Geometry: final body of the model. Coordinates: model frame, mm. Face numbers are marked on the shaded views. Give positions to 0.01 mm unless a question says otherwise; leave off trailing zeros. Loops run counter-clockwise (first coordinate to the right, second up) from the corner with the lowest first, then second, coordinate; pieces in that order, holes last.
from build123d import *

# Parameters (mm, degrees)
BALL_FACE_1_SKETCH_R       = 25
BALL_FACE_CUT_1_DEPTH      = 7.5
BALL_FACE_2_SKETCH_R       = 25
BALL_FACE_CUT_2_DEPTH      = 7.5
KEYED_BORE_20_REACH        = 210.153
SMALL_END_FLAT_CUT_1_REACH = 216.934
SMALL_START                = -9
SMALL_END_FLAT_CUT_2_REACH = 216.934
SMALL_START_2              = 9
SMALL_END_EYE_CUT_REACH    = 208.893
SMALL_END_EYE_SKETCH_R     = 9
HOLE_8_CUT_REACH           = 207.934
HOLE_8_CUT_END_RADIUS      = 25
HOLE_8_SKETCH_R            = 4


with BuildPart() as part:
    # Lever Profile Sketch → Lever Body Revolve (revolve)
    with BuildSketch(Plane(origin=(0, 0, 0), x_dir=(1, 0, 0), z_dir=(0, 1, 0)), mode=Mode.PRIVATE) as lever_body_revolve_sk:
        with BuildLine():
            Line((168.522248412, -10), (33.541019662, -10))
            ThreePointArc((33.541019662, -10), (25.376053853, -11.742581416), (18.633899812, -16.666666667))
            ThreePointArc((18.633899812, -16.666666667), (-8.920552244, -23.354308974), (-25, 0))
            Line((-25, 0), (203.66060556, 0))
            ThreePointArc((203.66060556, 0), (193.547273819, -15.542644572), (175.240158467, -12.592592593))
            ThreePointArc((175.240158467, -12.592592593), (172.122659912, -10.670635765), (168.522248412, -10))
        make_face()
    revolve(lever_body_revolve_sk.sketch.rotate(Axis((248.139692176, 0, 0), (-1, 0, 0)), 180), axis=Axis((248.139692176, 0, 0), (-1, 0, 0)))

    # Ball Face 1 Sketch → Ball Face Cut 1 (cut)
    with BuildSketch(Plane.XY.offset(25)):
        Circle(BALL_FACE_1_SKETCH_R)
    extrude(amount=-BALL_FACE_CUT_1_DEPTH, mode=Mode.SUBTRACT)


with BuildPart() as ball_face_cut_1_kept_piece:
    # of the separate pieces the step leaves, the one the design keeps (ball_face_cut_1_pieces_kept)
    add(part.part.solids().sort_by_distance((175.240158467, 0, -12.592592593))[0])

    # Ball Face 2 Sketch → Ball Face Cut 2 (cut)
    with BuildSketch(Plane.XY.offset(-25)):
        Circle(BALL_FACE_2_SKETCH_R)
    extrude(amount=BALL_FACE_CUT_2_DEPTH, mode=Mode.SUBTRACT)

    # Keyed Bore Sketch → Keyed Bore _20 (cut, up to next)
    with BuildSketch(Plane(origin=(0, 0, -17.5), x_dir=(-1, 0, 0), z_dir=(0, 0, -1)), mode=Mode.PRIVATE) as keyed_bore_20_sk1:
        with BuildLine():
            Line((-13, 2), (-9.797958971, 2))
            ThreePointArc((-9.797958971, 2), (10, 0), (-9.797958971, -2))
            Line((-9.797958971, -2), (-13, -2))
            Line((-13, -2), (-13, 2))
        make_face()
    keyed_bore_20_tool1 = extrude(keyed_bore_20_sk1.sketch, amount=-KEYED_BORE_20_REACH, mode=Mode.PRIVATE) & ball_face_cut_1_kept_piece.part
    add(keyed_bore_20_tool1.solids().sort_by_distance((0.430928, 0, -17.5))[0], mode=Mode.SUBTRACT)

    # Small End Flats Sketch → Small End Flat Cut 1 (cut, up to next)
    with BuildSketch(Plane.XY.offset(SMALL_START), mode=Mode.PRIVATE) as small_end_flat_cut_1_sk1:
        with BuildLine():
            Line((170.41252875, 5), (148.66060556, 5))
            Line((148.66060556, 5), (148.66060556, -5))
            Line((148.66060556, -5), (170.41252875, -5))
            ThreePointArc((170.41252875, -5), (203.66060556, 0), (170.41252875, 5))
        make_face()
    small_end_flat_cut_1_tool1 = extrude(small_end_flat_cut_1_sk1.sketch, amount=-SMALL_END_FLAT_CUT_1_REACH, mode=Mode.PRIVATE) & ball_face_cut_1_kept_piece.part
    add(small_end_flat_cut_1_tool1.solids().sort_by_distance((181.469026, 0, -9))[0], mode=Mode.SUBTRACT)

    # Sketch11_2 → Small End Flat Cut 2 (cut, up to next)
    with BuildSketch(Plane.XY.offset(SMALL_START_2), mode=Mode.PRIVATE) as small_end_flat_cut_2_sk1:
        with BuildLine():
            Line((170.41252875, 5), (148.66060556, 5))
            Line((148.66060556, 5), (148.66060556, -5))
            Line((148.66060556, -5), (170.41252875, -5))
            ThreePointArc((170.41252875, -5), (203.66060556, 0), (170.41252875, 5))
        make_face()
    small_end_flat_cut_2_tool1 = extrude(small_end_flat_cut_2_sk1.sketch, amount=SMALL_END_FLAT_CUT_2_REACH, mode=Mode.PRIVATE) & ball_face_cut_1_kept_piece.part
    add(small_end_flat_cut_2_tool1.solids().sort_by_distance((181.469026, 0, 9))[0], mode=Mode.SUBTRACT)

    # Small End Eye Sketch → Small End Eye Cut (cut, up to next)
    with BuildSketch(Plane.XY.offset(9), mode=Mode.PRIVATE) as small_end_eye_cut_sk1:
        with Locations((186.66060556, 0)):
            Circle(SMALL_END_EYE_SKETCH_R)
    small_end_eye_cut_tool1 = extrude(small_end_eye_cut_sk1.sketch, amount=-SMALL_END_EYE_CUT_REACH, mode=Mode.PRIVATE) & ball_face_cut_1_kept_piece.part
    add(small_end_eye_cut_tool1.solids().sort_by_distance((186.660606, 0, 9))[0], mode=Mode.SUBTRACT)

    # Hole _8 Cut: up to this sphere (the profile starts inside it)
    hole_8_cut_end = Location((0, 0, 0)) * Sphere(HOLE_8_CUT_END_RADIUS, mode=Mode.PRIVATE)
    # Hole _8 Sketch → Hole _8 Cut (cut, up to the surface)
    with BuildSketch(Plane(origin=(0, 0, 0), x_dir=(0, 0, -1), z_dir=(1, 0, 0)), mode=Mode.PRIVATE) as hole_8_cut_sk1:
        Circle(HOLE_8_SKETCH_R)
    hole_8_cut_tool1 = extrude(hole_8_cut_sk1.sketch, amount=-HOLE_8_CUT_REACH, mode=Mode.PRIVATE) & hole_8_cut_end
    add(hole_8_cut_tool1.solids().sort_by_distance((0, 0, 0))[0], mode=Mode.SUBTRACT)


solid = ball_face_cut_1_kept_piece.part
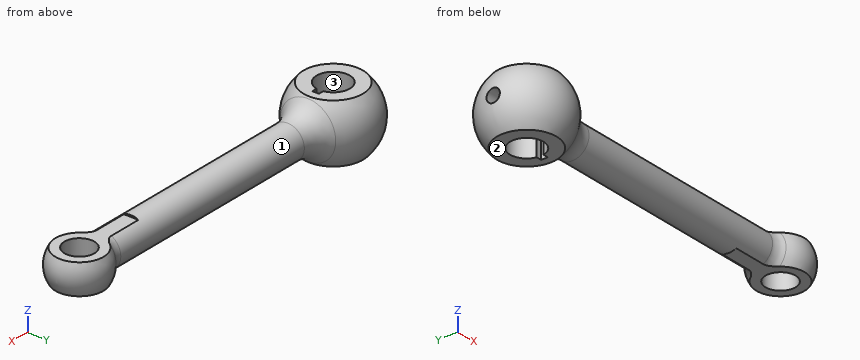
Item 1: Ray query, probe 1 along Z at (x, y) = (-14, 0); probe 2 along X at (y, z) = (-6.5, 7.5); probe 3 along Y at (x, z) = (0, -8). Return the intervals inside material, ascending.
Values follow:
probe 1: z = -17.5 to -4, 4 to 17.5
probe 2: x = -22.95 to -7.6, 7.6 to 180.44, 192.89 to 200.46
probe 3: y = -23.69 to -10, 10 to 23.69
Item 2: Draft query along Y for the marked faces 1, 2 and 3. Return one class per face: +Y half, -Y half, draft (parallel to the pull), parting line (faces both ways), or undercut.
Values follow:
face 1: parting line
face 2: draft
face 3: undercut
Item 3: Pin query (flat end, axial travel): pin 1 (23 mm diameter, centred on x = 177.5, y = 7, fed in from +Z); pin 2 (1 mm diameter, centred on x = 149.5, y = -8, fed in from -Z); pin 3 (12 mm diameter, centred on x = 80.5, z = 6.5, fed in from -Y). Return the tip coordinate at first contact, or that it passes through.
Values follow:
pin 1: stops at z = 9
pin 2: stops at z = -6.61
pin 3: stops at y = -9.99
Item 4: Section query B-B on x = 0. Return loops of the section in (y, z).
Values follow:
outline: (-17.85, -17.5) - (-10, -17.5) - (-10, 17.5) - (-17.85, 17.5) arc R25 ccw to start; (10, -17.5) - (17.85, -17.5) arc R25 ccw to (17.85, 17.5) - (10, 17.5) - close
Item 5: Section query C-C on z = 0. Return loops of the section in (x, y), plus the area to 3 significant figures.
Values follow:
outline: (-24.68, -4) arc R25 ccw to (18.63, -16.67) arc R20 cw to (33.54, -10) - (168.52, -10) arc R10 cw to (175.24, -12.59) arc R17 ccw (long way) to (175.24, 12.59) arc R10 cw to (168.52, 10) - (33.54, 10) arc R20 cw to (18.63, 16.67) arc R25 ccw to (-24.68, 4) - (-9.17, 4) arc R10 cw to (9.8, 2) - (13, 2) - (13, -2) - (9.8, -2) arc R10 cw to (-9.17, -4) - close; hole circle Ø18 at (186.66, 0)
area: 5,130 mm2
Item 6: Section query D-D on x = 111. Return loops of the section in (y, z).
Values follow:
outline: circle Ø20 at (0, 0)
Item 7: Section query A-A on y = 0. Return loops of the section in (x, z).
Values follow:
outline: (-24.68, -4) arc R25 ccw to (-17.85, -17.5) - (-10, -17.5) - (-10, -4) - close; (-24.68, 4) - (-10, 4) - (-10, 17.5) - (-17.85, 17.5) arc R25 ccw to start; (13, -17.5) - (17.85, -17.5) arc R25 ccw to (18.63, -16.67) arc R20 cw to (33.54, -10) - (148.66, -10) - (148.66, -9) - (177.66, -9) - (177.66, 9) - (148.66, 9) - (148.66, 10) - (33.54, 10) arc R20 cw to (18.63, 16.67) arc R25 ccw to (17.85, 17.5) - (13, 17.5) - close; (195.66, -9) - (201.08, -9) arc R17 ccw to (201.08, 9) - (195.66, 9) - close
